The listing builds one solid part. Answer for the finished solid, in the listing's coordinates (mm). Round coordinates to 2 decimals unless told otherwise and drop trailing zeros. Order: outer loops, then holes, each group sorted by start corner. A loop starts at its lowest first (then second) coordinate and runs counter-clockwise, first axis right, second up. Notation, with made-up numbers: M 68.25,12.25 L 85.25,12.25 A23 ccw 85.25,49.25 Z; hole C 89.25,-20.75 d1. An arc over 180 degrees is marked long. Put each result on its own line as item: value. Start each with the question number.
1. The part is cut by section A-A (z = 1.6). Give the vertices of the cut face in (x, y), then the cut area to 3 significant figures.
2. Consider line 1 (X direction, y = -59.5, z = 1.95); line 2 (Y direction, x = -72.75, z = 0.85); line 3 (X direction, y = -36, z = 0.1). Determine where each line is inside the solid, lowest interval first.
3. This flat-tipped pin is pushed along its axis until it touches: pin 1 Ø1.5 at (x, y) = (-73.19, -40.19) entering from -Z. Where does it stop, or does it pass through?
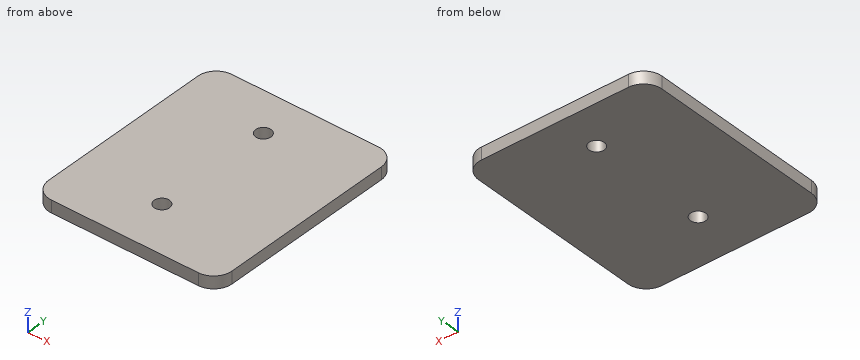
from build123d import *

# Parameters (mm, degrees)
SKETCH1_W           = 30
SKETCH1_H           = 35
BOSS_EXTRUDE1_DEPTH = 2
FILLET1_R           = 3
M3_TAPPED_HOLE1_D   = 2.5


with BuildPart() as part:
    # Sketch1 → Boss-Extrude1 (new body)
    with BuildSketch(Plane.XY):
        with Locations((-72.289490021, -50.654966575)):
            Rectangle(SKETCH1_W, SKETCH1_H)
    extrude(amount=BOSS_EXTRUDE1_DEPTH)

    # Fillet1
    fillet1_edges = [part.edges().sort_by_distance(p)[0] for p in [
        (-87.289490021, -33.154966575, 1),
        (-57.289490021, -33.154966575, 1),
        (-57.289490021, -68.154966575, 1),
        (-87.289490021, -68.154966575, 1),
    ]]
    fillet(fillet1_edges, radius=FILLET1_R)

    # M3 Tapped Hole1 (through all)
    with Locations(Plane.XY.offset(2)):
        with Locations((-73.189490021, -59.894365688), (-73.189490021, -40.194365688)):
            Hole(M3_TAPPED_HOLE1_D / 2)


solid = part.part
Resolved:
1. outline: M -87.29,-65.15 A3 ccw -84.29,-68.15 L -60.29,-68.15 A3 ccw -57.29,-65.15 L -57.29,-36.15 A3 ccw -60.29,-33.15 L -84.29,-33.15 A3 ccw -87.29,-36.15 Z; hole C -73.19,-59.89 d2.5; hole C -73.19,-40.19 d2.5
1. area: 1,030 mm2
2. line 1: -87.29 to -74.38, -72 to -57.29
2. line 2: -68.15 to -61.06, -58.72 to -41.36, -39.02 to -33.15
2. line 3: -87.29 to -57.29
3. pin 1: through
